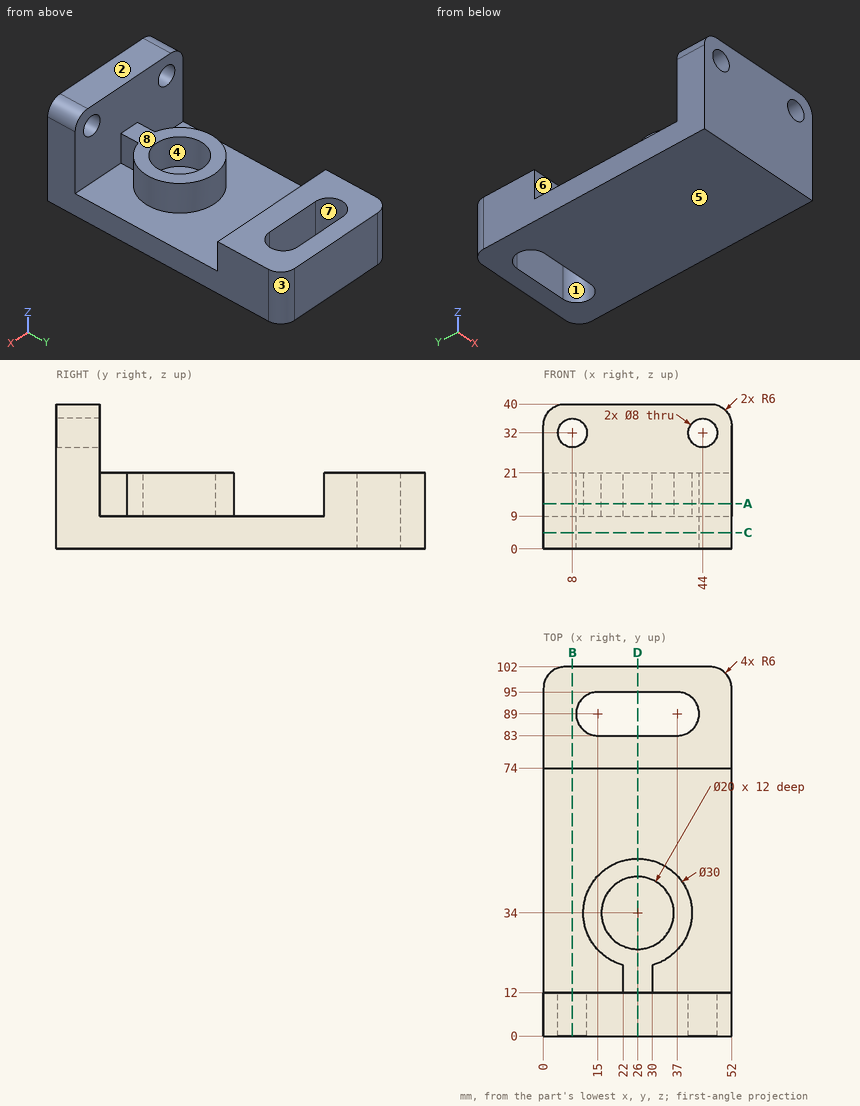
Part print with two shaded views. Sizes in mm from the minimum x, y, z corner. A direction names the side the tool comes from. Round coordinates to 2 decimals unless told otherwise and drop trailing zeros. Write each loop counter-clockwise with the first axis right and the second up, starting at its lowest first coordinate (ties: lowest second). Pieces come first, ordered by that corner, then holes. Notation, with made-up numbers: (49, 60.25) - (107, 60.25) arc R12 ccw to (107, 79.25) - close; hole circle Ø1 at (72.5, 27.5). An arc over 180 degrees is marked (long way). Answer as CSV lines item,"result".
Q1. Tool access for the marked faces 4, 5, 6, 7 and 8: list every direction of +Z, -Z, +X, -X, +Y, -Y with a clear straight run to the whole face (end or side of a thin tool).
Report:
face 4,"+Z"
face 5,"-Z, +X, -X, +Y, -Y"
face 6,"+Z, +X, -X"
face 7,"+Z, -Z"
face 8,"+Z, +X, -X, +Y"
Q2. Drill centre lines: probe 1 along X at (y, z) = (3.75, 32); probe 2 along Y at (x, z) = (19, 13); probe 3 along Y at (x, z) = (9.5, 15). Where is each one in solid material? Low to high. Write a range as [from, to].
Report:
probe 1,"x = [0, 4], [12, 40], [48, 52]"
probe 2,"y = [0, 12], [20.73, 26.86], [41.14, 47.27], [74, 83], [95, 102]"
probe 3,"y = [0, 12], [74, 86.6], [91.4, 102]"
Q3. Drop flat-ended pins along their axis: pin 1 (1.5 mm diameter, centred on x = 27.5, y = 32, fed in from -Z); pin 2 (6 mm diameter, centred on y = 16.5, z = 14.5, fed in from +X); pin 3 (1 mm diameter, centred on y = 32, z = 18.5, fed in from -X); pin 4 (2.5 mm diameter, centred on y = 15, z = 16.5, fed in from -X). Give the stop position or say it passes through.
Report:
pin 1,"stops at z = 0"
pin 2,"stops at x = 30"
pin 3,"stops at x = 11.08"
pin 4,"stops at x = 22"
Q4. Pull direction Y, two halves, no side cores. Call the marked faces 1, 2 and 3: +Y half, -Y half, draft (parallel to the pull), parting line (faces both ways), or undercut.
Report:
face 1,"undercut"
face 2,"draft"
face 3,"+Y half"
Q5. Cut at C-C (z = 4.5). Write the cut outline in (x, y).
Report:
outline,"(0, 0) - (52, 0) - (52, 96) arc R6 ccw to (46, 102) - (6, 102) arc R6 ccw to (0, 96) - close; hole (15, 83) - (37, 83) arc R6 ccw to (37, 95) - (15, 95) arc R6 ccw to start"
Q6. Cut at A-A (z = 12.5). Write the cut outline in (x, y), and give its area (3 significant figures).
Report:
outline,"(0, 0) - (52, 0) - (52, 12) - (30, 12) - (30, 19.54) arc R15 ccw (long way) to (22, 19.54) - (22, 12) - (0, 12) - close; (0, 74) - (52, 74) - (52, 96) arc R6 ccw to (46, 102) - (6, 102) arc R6 ccw to (0, 96) - close; hole (15, 83) - (37, 83) arc R6 ccw to (37, 95) - (15, 95) arc R6 ccw to start; hole circle Ø20 at (26, 34)"
area,"2,140 mm^2"
Q7. Cut at D-D (x = 26). Write the cut outline in (y, z).
Report:
outline,"(0, 0) - (83, 0) - (83, 21) - (74, 21) - (74, 9) - (49, 9) - (49, 21) - (44, 21) - (44, 9) - (24, 9) - (24, 21) - (12, 21) - (12, 40) - (0, 40) - close; (95, 0) - (102, 0) - (102, 21) - (95, 21) - close"
Q8. Cut at B-B (x = 8). Write the cut outline in (y, z).
Report:
outline,"(0, 0) - (102, 0) - (102, 21) - (74, 21) - (74, 9) - (12, 9) - (12, 28) - (0, 28) - close; (0, 36) - (12, 36) - (12, 40) - (0, 40) - close"
